```python
from build123d import *

# Parameters (mm, degrees)
SKETCH8_R                  = 22.5
BOSS_EXTRUDE2_DEPTH        = 25
M30X2_0_TAPPED_HOLE1_D     = 28
M30X2_0_TAPPED_HOLE1_DEPTH = 70
M30X2_0_TAPPED_HOLE1_TIP   = 8.412048666
BOSS_EXTRUDE3_START        = 2.5
SKETCH11_R                 = 20
SKETCH11_R_2               = 14
BOSS_EXTRUDE3_DEPTH        = 2.5
CHAMFER1_SIZE              = 1


with BuildPart() as part:
    # Sketch8 → Boss-Extrude2 (new body)
    with BuildSketch(Plane.XY):
        with Locations((-69.420997024, 0)):
            Circle(SKETCH8_R)
    extrude(amount=BOSS_EXTRUDE2_DEPTH)

    # M30x2.0 Tapped Hole1
    with Locations(Plane(origin=(-69.420997024, 0, 25), x_dir=(1, 0, 0), z_dir=(0, 0, 1))):
        with Locations((0, 0)):
            Hole(M30X2_0_TAPPED_HOLE1_D / 2, depth=M30X2_0_TAPPED_HOLE1_DEPTH)
            with Locations((0, 0, -(M30X2_0_TAPPED_HOLE1_DEPTH + M30X2_0_TAPPED_HOLE1_TIP / 2))):  # 118° drill point
                Cone(0, M30X2_0_TAPPED_HOLE1_D / 2, M30X2_0_TAPPED_HOLE1_TIP, mode=Mode.SUBTRACT)

    # Sketch11 → Boss-Extrude3 (add)
    with BuildSketch(Plane(origin=(0, 0, 0), x_dir=(-1, 0, 0), z_dir=(0, 0, -1)).offset(BOSS_EXTRUDE3_START)):
        with Locations(Location((69.420997024, 0, 0), (0, 0, 180))):
            Circle(SKETCH11_R)
        with Locations(Location((69.420997024, 0, 0), (0, 0, 180))):
            Circle(SKETCH11_R_2, mode=Mode.SUBTRACT)
    extrude(amount=-BOSS_EXTRUDE3_DEPTH)

    # Chamfer1
    chamfer1_edges = [part.edges().sort_by_distance(p)[0] for p in [
        (-91.920997024, 0, 0),
        (-91.920997024, 0, 25),
        (-55.420997024, 0, 25),
    ]]
    chamfer(chamfer1_edges, length=CHAMFER1_SIZE)


solid = part.part
```
Source: CAD feature listing. Evaluate the final solid. Frame: model axes, mm. A direction names the side the tool comes from. Coordinates: 2 decimals unless noted, no trailing zeros. Write each loop counter-clockwise with the first axis right and the second up, starting at its lowest first coordinate (ties: lowest second). Pieces come first, ordered by that corner, then holes. Notation, with made-up numbers: M -21,-1 L 13,-1 A24 cw 13,23 Z; hole C -22.5,-8.5 d2. An arc over 180 degrees is marked long. Answer as a JSON object with one key per item and string values.
1. Contact query for flat-ended pins moving along their axis: P1, Ø4, axis at x = -71, z = 3, coming from the -Y side; P2, Ø10, axis at y = -5.5, z = 8.5, coming from the +X side; P3, Ø4, axis at x = -58.5, z = 6, coming from the +Y side; P4, Ø1.5, axis at x = -85, y = -17.5, coming from the -Z side. Output: stop coordinate, or through.
Evaluation:
{"P1": "y = -22.5", "P2": "x = -46.93", "P3": "y = 20.66", "P4": "through"}
2. Access query for faces 1 (the flat face through (-84.1, -4.5, 25)), 2 (the flat face through (-50, -6, 0)). Directions: +Z, -Z, +X, -X, +Y, -Y. A direction counts if a zero-diameter tool reaches every point of the face in a straight line with its end or side. Return the directions, or none.
Evaluation:
{"face 1": "+Z, +X, -X, +Y, -Y", "face 2": "-Z"}
3. Cut plane A-A on y = 0. Output: boundary loops of the cut face in (x, z), plus the area to 3 significant figures.
Evaluation:
{"outline": "M -91.92,1 L -90.92,0 L -89.42,0 L -89.42,-2.5 L -83.42,-2.5 L -83.42,24 L -84.42,25 L -90.92,25 L -91.92,24 Z; M -55.42,-2.5 L -49.42,-2.5 L -49.42,0 L -47.92,0 L -46.92,1 L -46.92,24 L -47.92,25 L -54.42,25 L -55.42,24 Z", "area": "452 mm^2"}
4. Cut plane B-B on z = 9.75. Output: boundary loops of the cut face in (x, y).
Evaluation:
{"outline": "C -69.42,0 d45; hole C -69.42,0 d28"}
5. Ray query, L1, parallel to Y at x = -62, z = 2; L2, parallel to X at y = -11.5, z = 22.25; L3, parallel to X at y = 3.5, z = 20. Return the intervals inside material, ascending.
Evaluation:
{"L1": "-21.24 to -11.87, 11.87 to 21.24", "L2": "-88.76 to -77.41, -61.44 to -50.08", "L3": "-91.65 to -82.98, -55.87 to -47.19"}
